Build history of the part. All positions in model axes, mm. Round coordinates to 2 decimals unless told otherwise and drop trailing zeros. Loops run counter-clockwise (first coordinate to the right, second up) from the corner with the lowest first, then second, coordinate; pieces in that order, holes last.
from build123d import *

# Parameters (mm, degrees)
SKETCH_1_W             = 120
SKETCH_1_H             = 35
EXTRUDE_1_DEPTH        = 10
HOLE_WIZARD_M4_1_D     = 3.3
SKETCH_5_R             = 2.25
CUT_EXTRUDE_1_DEPTH    = 28
CHAMFER_1_SIZE         = 2
PATTERN_LINEAR_1_COUNT = 2
PATTERN_LINEAR_1_PITCH = 17.5


with BuildPart() as part:
    # 草图1 → 凸台-拉伸1 (new body)
    with BuildSketch(Plane(origin=(0, 0, 0), x_dir=(0, 0, -1), z_dir=(1, 0, 0))):
        Rectangle(SKETCH_1_W, SKETCH_1_H)
    extrude(amount=EXTRUDE_1_DEPTH)

    # M4 螺纹孔1 (through all)
    with Locations(Plane.ZY):
        with Locations((45, 5), (45, -5)):
            Hole(HOLE_WIZARD_M4_1_D / 2)

    # 草图5 → 切除-拉伸1 (cut)
    with BuildSketch(Plane.ZY):
        with Locations((-47.5, 9)):
            Circle(SKETCH_5_R)
        with Locations(Location((-47.5, -9, 0), (0, 0, 180))):
            Circle(SKETCH_5_R)
    cut_extrude_1 = extrude(amount=-CUT_EXTRUDE_1_DEPTH, mode=Mode.SUBTRACT)

    # 倒角1
    chamfer_1_edges = [part.edges().sort_by_distance(p)[0] for p in [
        (5, -17.5, 60),
        (5, 17.5, 60),
    ]]
    chamfer(chamfer_1_edges, length=CHAMFER_1_SIZE)

    # 阵列(线性)1: 切除-拉伸1 ×2
    with Locations(*[(0, 0, i * PATTERN_LINEAR_1_PITCH) for i in range(1, PATTERN_LINEAR_1_COUNT)]):
        add(cut_extrude_1, mode=Mode.SUBTRACT)


solid = part.part
(1) Slice it at A-A on z = 45. List the corners of the cut face in (x, y).
Responses:
outline: (0, -17.5) - (10, -17.5) - (10, -6.65) - (0, -6.65) - close; (0, -3.35) - (10, -3.35) - (10, 3.35) - (0, 3.35) - close; (0, 6.65) - (10, 6.65) - (10, 17.5) - (0, 17.5) - close
(2) Probe line 1 (Y direction, x = 3, z = -30); line 2 (Y direction, x = 3, z = 45); line 3 (Z direction, x = 6.75, y = -9). List the from-to ranges inside material, lowest first.
Responses:
line 1: y = -17.5 to -11.25, -6.75 to 6.75, 11.25 to 17.5
line 2: y = -17.5 to -6.65, -3.35 to 3.35, 6.65 to 17.5
line 3: z = -60 to -49.75, -45.25 to -32.25, -27.75 to 60
(3) Slice it at C-C on x = 3.75. List the corners of the cut face in (y, z), plus the area to 3 significant figures.
Responses:
outline: (-17.5, -60) - (17.5, -60) - (17.5, 58) - (15.5, 60) - (-15.5, 60) - (-17.5, 58) - close; hole circle Ø4.5 at (-9, -47.5); hole circle Ø4.5 at (-9, -30); hole circle Ø3.3 at (-5, 45); hole circle Ø3.3 at (5, 45); hole circle Ø4.5 at (9, -47.5); hole circle Ø4.5 at (9, -30)
area: 4,120 mm2
(4) Slice it at B-B on y = -9. List the corners of the cut face in (x, z).
Responses:
outline: (0, -60) - (10, -60) - (10, -49.75) - (0, -49.75) - close; (0, -45.25) - (10, -45.25) - (10, -32.25) - (0, -32.25) - close; (0, -27.75) - (10, -27.75) - (10, 60) - (0, 60) - close
(5) Pull direction Y, two halves, no side cores. Call faces 1 (the face through (5, 0, -60)), 2 (the face through (5, -17.5, 0)), 3 (the face through (5, 17.5, 0)), 4 (the face through (5.07, 5.07, 46.65)): +Y half, -Y half, draft (parallel to the pull), parting line (faces both ways), or undercut.
Responses:
face 1: draft
face 2: -Y half
face 3: +Y half
face 4: undercut
